```python
from build123d import *


with BuildPart() as part:
    # 草图1 → 旋转2 (revolve)
    with BuildSketch(Plane(origin=(0, 0, 0), x_dir=(0, 0, -1), z_dir=(1, 0, 0)), mode=Mode.PRIVATE) as revolve_2_sk:
        with BuildLine():
            Line((0, 15), (0, 7.5))
            Line((0, 7.5), (5, 7.5))
            Line((5, 7.5), (5, 9))
            ThreePointArc((5, 9), (4, 10), (3, 9))
            Line((3, 9), (1.5, 9))
            Line((1.5, 9), (1.5, 13.5))
            Line((1.5, 13.5), (5, 13.5))
            Line((5, 13.5), (5, 15))
            Line((5, 15), (0, 15))
        make_face()
    revolve_2 = revolve(revolve_2_sk.sketch.rotate(Axis((0, 0, 4.217424625), (0, 0, -1)), 90), axis=Axis((0, 0, 4.217424625), (0, 0, -1)))

    # 镜向2: 旋转2 across plane
    add(revolve_2.mirror(Plane(origin=(0, 15, 0), x_dir=(1, 0, 0), z_dir=(0, 0, -1))))


solid = part.part
```
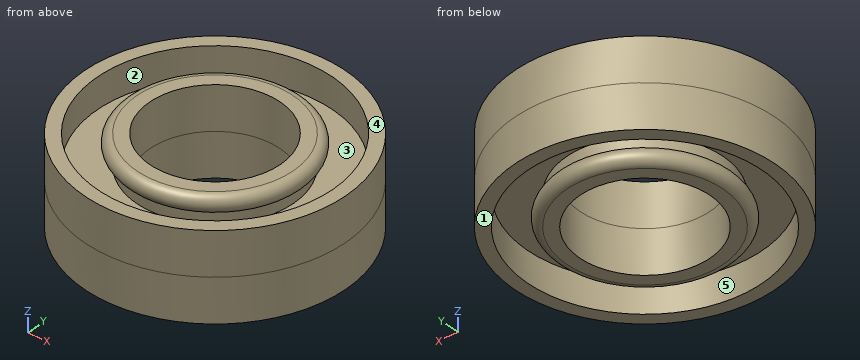
Input: part model. Units: mm. Frame: model coordinates. Face numbers are marked on the shaded views. A direction names the side the tool comes from. Round coordinates to 2 decimals unless told otherwise and drop trailing zeros. Write each loop counter-clockwise with the first axis right and the second up, starting at its lowest first coordinate (ties: lowest second). Pieces come first, ordered by that corner, then holes. Notation, with made-up numbers: (57, 70) - (71, 70) arc R14 cw to (71, 89) - close; hole circle Ø6 at (6.5, 54.5). An arc over 180 degrees is marked (long way). Write item = value, one per line.
(1) Contact query for flat-ended pins moving along their axis: pin 1 Ø8 at (x, y) = (3.5, 5.5) entering from +Z; pin 2 Ø12 at (x, y) = (0, 0) entering from -Z; pin 3 Ø4 at (x, z) = (2.5, -0.5) entering from +Y; pin 4 Ø1.5 at (x, z) = (2.5, -1) entering from -Y. Output: stop coordinate, or through.
Geometry check:
pin_1 = 5
pin_2 = through
pin_3 = 14.99
pin_4 = -14.9
(2) Section query A-A on y = 0. Output: boundary loops of the cut face in (x, z), then the cut area to 3 significant figures.
Geometry check:
outline = (-15, -5) - (-13.5, -5) - (-13.5, -1.5) - (-9, -1.5) - (-9, -3) arc R1 ccw to (-9, -5) - (-7.5, -5) - (-7.5, 5) - (-9, 5) arc R1 ccw to (-9, 3) - (-9, 1.5) - (-13.5, 1.5) - (-13.5, 5) - (-15, 5) - close; (7.5, -5) - (9, -5) arc R1 ccw to (9, -3) - (9, -1.5) - (13.5, -1.5) - (13.5, -5) - (15, -5) - (15, 5) - (13.5, 5) - (13.5, 1.5) - (9, 1.5) - (9, 3) arc R1 ccw to (9, 5) - (7.5, 5) - close
area = 93.3 mm^2
(3) Pull-direction query (Y, two-part tool) for the marked faces 4 and 5; classes: +Y half, -Y half, draft (parallel to the pull), parting line (faces both ways), or undercut.
Geometry check:
face_4 = draft
face_5 = undercut
(4) Material intervals for probe 1 along Y at (x, z) = (0, -2.6); probe 2 along X at (y, z) = (3.5, 2.25); probe 3 along Y at (x, z) = (0, -3.15), sorted ascending.
Geometry check:
probe_1 = -15 to -13.5, -9 to -7.5, 7.5 to 9, 13.5 to 15
probe_2 = -14.59 to -13.04, -8.29 to -6.63, 6.63 to 8.29, 13.04 to 14.59
probe_3 = -15 to -13.5, -9.53 to -7.5, 7.5 to 9.53, 13.5 to 15
(5) Section query C-C on x = -10.5. Output: boundary loops of the cut face in (y, z).
Geometry check:
outline = (-10.71, -5) - (-8.49, -5) - (-8.49, -1.5) - (8.49, -1.5) - (8.49, -5) - (10.71, -5) - (10.71, 5) - (8.49, 5) - (8.49, 1.5) - (-8.49, 1.5) - (-8.49, 5) - (-10.71, 5) - close
(6) Access query for the marked faces 1, 2 and 3. Directions: +Z, -Z, +X, -X, +Y, -Y. A direction counts if a zero-diameter tool reaches every point of the face in a straight line with its end or side. Return the directions, or none.
Geometry check:
face_1 = -Z, +X, -X, +Y, -Y
face_2 = +Z
face_3 = none
